Work out the finished part from the listing and answer in its coordinate system (mm). A direction names the side the tool comes from. Give positions to 0.01 mm unless a question says otherwise; leave off trailing zeros. Order: outer loops, then holes, each group sorted by start corner. A loop starts at its lowest first (then second) coordinate and runs counter-clockwise, first axis right, second up. Notation, with made-up numbers: M -3,-36 L 23,-36 A17 ccw 23,-24 Z; hole C 14.5,-29.5 d4. An arc over 180 degrees is marked long. One line per item, written item: value.
from build123d import *

# Parameters (mm, degrees)
SKETCH1_W           = 110
SKETCH1_H           = 200
SKETCH1_R           = 3.25
BOSS_EXTRUDE1_DEPTH = 10
SKETCH2_W           = 77.344894784
SKETCH2_H           = 153.75567248
BOSS_EXTRUDE2_DEPTH = 730
SKETCH4_W           = 110
SKETCH4_H           = 200
SKETCH4_R           = 3.25
BOSS_EXTRUDE4_DEPTH = 10


with BuildPart() as part:
    # Sketch1 → Boss-Extrude1 (new body)
    with BuildSketch(Plane(origin=(0, 0, 0), x_dir=(1, 0, 0), z_dir=(0, 1, 0))):
        Rectangle(SKETCH1_W, SKETCH1_H)
        with Locations(Location((-47, 92, 0), (0, 0, 270))):
            Circle(SKETCH1_R, mode=Mode.SUBTRACT)
        with Locations(Location((47, 92, 0), (0, 0, 270))):
            Circle(SKETCH1_R, mode=Mode.SUBTRACT)
        with Locations(Location((47, -92, 0), (0, 0, 270))):
            Circle(SKETCH1_R, mode=Mode.SUBTRACT)
        with Locations(Location((-47, -92, 0), (0, 0, 270))):
            Circle(SKETCH1_R, mode=Mode.SUBTRACT)
    extrude(amount=BOSS_EXTRUDE1_DEPTH)

    # Sketch2 → Boss-Extrude2 (add)
    with BuildSketch(Plane(origin=(0, 10, 0), x_dir=(1, 0, 0), z_dir=(0, 1, 0))):
        Rectangle(SKETCH2_W, SKETCH2_H)
    extrude(amount=BOSS_EXTRUDE2_DEPTH)

    # Sketch4 → Boss-Extrude4 (add)
    with BuildSketch(Plane(origin=(0, 740, 0), x_dir=(1, 0, 0), z_dir=(0, 1, 0))):
        Rectangle(SKETCH4_W, SKETCH4_H)
        with Locations(Location((-47, 92, 0), (0, 0, 270))):
            Circle(SKETCH4_R, mode=Mode.SUBTRACT)
        with Locations(Location((47, 92, 0), (0, 0, 270))):
            Circle(SKETCH4_R, mode=Mode.SUBTRACT)
        with Locations(Location((47, -92, 0), (0, 0, 270))):
            Circle(SKETCH4_R, mode=Mode.SUBTRACT)
        with Locations(Location((-47, -92, 0), (0, 0, 270))):
            Circle(SKETCH4_R, mode=Mode.SUBTRACT)
    extrude(amount=BOSS_EXTRUDE4_DEPTH)


solid = part.part
(1) Section A-A, the plane x = 11.5 is taken. Give the vertices of the cut face in (y, z).
Findings:
outline: M 0,-100 L 10,-100 L 10,-76.88 L 740,-76.88 L 740,-100 L 750,-100 L 750,100 L 740,100 L 740,76.88 L 10,76.88 L 10,100 L 0,100 Z
(2) Find the intervals of material crossed by probe 1 along X at (y, z) = (746, 92); probe 2 along Y at (x, z) = (40, -61); probe 3 along Z at (x, y) = (-3, 100), in increasing order. Write a range as from..to.
Findings:
probe 1: x = -55..-50.25, -43.75..43.75, 50.25..55
probe 2: y = 0..10, 740..750
probe 3: z = -76.88..76.88
(3) Section C-C, the plane y = 317.5 is taken. Give the vertices of the cut face in (x, z), then the cut area to 3 significant figures.
Findings:
outline: M -38.67,-76.88 L 38.67,-76.88 L 38.67,76.88 L -38.67,76.88 Z
area: 11,900 mm^2
(4) Section B-B, the plane z = 48 is taken. Give the vertices of the cut face in (x, y), then the cut area to 3 significant figures.
Findings:
outline: M -55,0 L 55,0 L 55,10 L 38.67,10 L 38.67,740 L 55,740 L 55,750 L -55,750 L -55,740 L -38.67,740 L -38.67,10 L -55,10 Z
area: 58,700 mm^2
(5) Given P1, Ø6, axis at y = 466, z = -41.5, coming from the +X side; P2, Ø1.5, axis at y = 486.5, z = 26.5, coming from the -X side; P3, Ø1.5, axis at x = -4.5, y = 460.5, coming from the -Z side; P4, Ø6, axis at x = -47, z = -92, coming from the -Y side, each flat-ended and moving along its own axis, determine where each tip first touches the part or whether it passes through.
Findings:
P1: stops at x = 38.67
P2: stops at x = -38.67
P3: stops at z = -76.88
P4: passes through
(6) Which of the six approach directions +Z, -Z, +X, -X, +Y, -Y give full straight-line access (tool end or side, diameter ignored) to faces 1 (the flat face through (-38.672, 370, 1)), 2 (the flat face through (-1, 370, -76.878)), 3 (the flat face through (-50, 740, -1)), 4 (the flat face through (-1, 370, 76.878)), 5 (the flat face through (38.672, 370, 1))?
Findings:
face 1: +Z, -Z, -X
face 2: -Z, +X, -X
face 3: none
face 4: +Z, +X, -X
face 5: +Z, -Z, +X
